```python
from build123d import *

# Parameters (mm, degrees)
EYE_START                  = 22.5
EYE_LUG_SKETCH_R           = 7
EYE_LUG_DEPTH              = 7.5
EYE_START_2                = 2.5
EYE_BOSS_SKETCH_R          = 14
EYE_BOSS_SKETCH_R_2        = 7
EYE_BOSS_28_DEPTH          = 2.5
WEB_RIB_6MM_REACH          = 108.099
WEB_RIB_SKETCH_WALL_W      = 244.198020726
WEB_RIB_SKETCH_WALL_H      = 6
CROSS_BORE_SKETCH_R        = 8
CROSS_BORE_16_DEPTH        = 51.5
TAPPED_HOLE_M12_D          = 10.2
BARREL_SLOT_CUT_DEPTH      = 107.099010428
BARREL_SLOT_CUT_DEPTH_BACK = 107.099010428
BARREL_SLOT_SKETCH_W       = 10
BARREL_SLOT_SKETCH_H       = 8


with BuildPart() as part:
    # Barrel Profile Sketch → Cylinder Barrel (revolve)
    with BuildSketch(Plane.XY, mode=Mode.PRIVATE) as cylinder_barrel_sk:
        Polygon((-39, 11), (-39, 30), (39, 30), (39, 11), (17.5, 11), (17.5, 18), (-17.5, 18), (-17.5, 11), align=None)
    revolve(cylinder_barrel_sk.sketch.rotate(Axis((-46.634042553, 0, 0), (1, 0, 0)), 90), axis=Axis((-46.634042553, 0, 0), (1, 0, 0)))

    # Eye Lug Sketch → Eye Lug (add)
    with BuildSketch(Plane(origin=(0, 0, 0), x_dir=(0, 0, -1), z_dir=(1, 0, 0)).offset(EYE_START)):
        with BuildLine():
            Line((-29.393876913, 6), (-13.71714256, 82.8))
            ThreePointArc((-13.71714256, 82.8), (0, 94), (13.71714256, 82.8))
            Line((13.71714256, 82.8), (29.393876913, 6))
            ThreePointArc((29.393876913, 6), (0, 30), (-29.393876913, 6))
        make_face()
        with Locations((0, 80)):
            Circle(EYE_LUG_SKETCH_R, mode=Mode.SUBTRACT)
    eye_lug = extrude(amount=-EYE_LUG_DEPTH)

    # Eye Boss Sketch → Eye Boss Ø28 (add)
    with BuildSketch(Plane(origin=(22.5, 0, 0), x_dir=(0, 0, -1), z_dir=(1, 0, 0)).offset(EYE_START_2)):
        with Locations(Location((0, 80, 0), (0, 0, 168.463040967))):
            Circle(EYE_BOSS_SKETCH_R)
        with Locations((0, 80)):
            Circle(EYE_BOSS_SKETCH_R_2, mode=Mode.SUBTRACT)
    eye_boss_28 = extrude(amount=-EYE_BOSS_28_DEPTH)

    # Mirrored Eye Lug: Eye Lug, Eye Boss Ø28 across plane
    add(eye_lug.mirror(Plane(origin=(0, 0, 0), x_dir=(0, 0, 1), z_dir=(1, 0, 0))))
    add(eye_boss_28.mirror(Plane(origin=(0, 0, 0), x_dir=(0, 0, 1), z_dir=(1, 0, 0))))

    # Web Rib Sketch wall → Web Rib 6mm (add, up to next)
    with BuildSketch(Plane(origin=(0, 63.7, 0), x_dir=(1, 0, 0), z_dir=(0, 1, 0)), mode=Mode.PRIVATE) as web_rib_6mm_sk1:
        Rectangle(WEB_RIB_SKETCH_WALL_W, WEB_RIB_SKETCH_WALL_H)
    web_rib_6mm_tool1 = extrude(web_rib_6mm_sk1.sketch, amount=-WEB_RIB_6MM_REACH, mode=Mode.PRIVATE) - part.part
    add(web_rib_6mm_tool1.solids().sort_by_distance((0, 63.7, 0))[0])

    # Cross Bore Sketch → Cross Bore Ø16 (cut)
    with BuildSketch(Plane(origin=(0, 0, 0), x_dir=(1, 0, 0), z_dir=(0, 1, 0))):
        with Locations(Location((0, 0, 0), (0, 0, 270))):
            Circle(CROSS_BORE_SKETCH_R)
    extrude(amount=-CROSS_BORE_16_DEPTH, mode=Mode.SUBTRACT)

    # Tapped Hole M12 (through all)
    with Locations(Plane(origin=(0, 46.774811557, 3), x_dir=(1, 0, 0), z_dir=(0, 0, 1))):
        with Locations((0, 0)):
            Hole(TAPPED_HOLE_M12_D / 2)

    # Barrel Slot Sketch → Barrel Slot Cut (cut, two sides: drawn at the far end of the back side and taken through both)
    with BuildSketch(Plane.XY.offset(-BARREL_SLOT_CUT_DEPTH_BACK)):
        with Locations((-34, 26)):
            Rectangle(BARREL_SLOT_SKETCH_W, BARREL_SLOT_SKETCH_H)
        with Locations((34, 26)):
            Rectangle(BARREL_SLOT_SKETCH_W, BARREL_SLOT_SKETCH_H)
    extrude(amount=BARREL_SLOT_CUT_DEPTH + BARREL_SLOT_CUT_DEPTH_BACK, mode=Mode.SUBTRACT)


solid = part.part
```
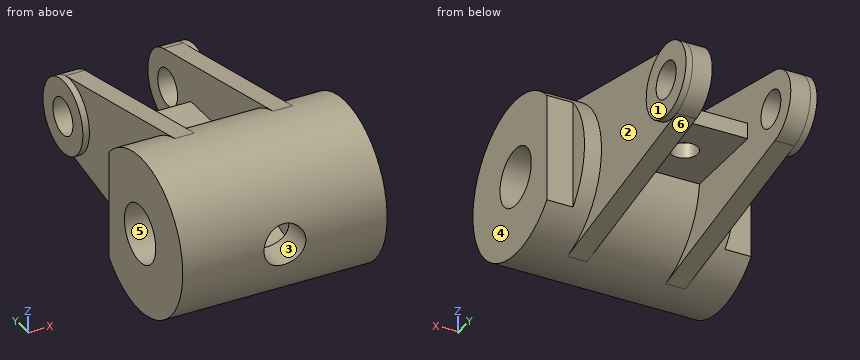
The listing builds one solid part. Answer for the finished solid, in the listing's coordinates (mm). Face numbers are marked on the shaded views. A direction names the side the tool comes from. Coordinates: 2 decimals unless noted, no trailing zeros. Loops run counter-clockwise (first coordinate to the right, second up) from the corner with the lowest first, then second, coordinate; pieces in that order, holes last. Notation, with made-up numbers: (-13.5, -39) -> (23.5, -39) arc R10 ccw to (23.5, -25) -> close; hole circle Ø11 at (26, -17.75). An arc over 180 degrees is marked (long way). Use one line per item in the form item = value. Start each with the question number.
Item 1: A tool of negligible diameter and unlimited length cuts with its end or side. For the marked faces 1, 2 and 3, from which of +Z, -Z, +X, -X, +Y, -Y can it reach the whole face along a straight path? Write none if from no direction.
Item 2: The part is cut by section D-D on x = 11. Determine the outline of the cut face in (y, z), then the cut area to 3 significant figures.
Item 3: The mould has two halves that part along Y. Classify the marked faces 4, 5 and 6: released by +Y, released by -Y, zero draft, split by the parting line, or undercut.
Item 4: Consider L1, parallel to X at y = 76.5, z = -7; L2, parallel to X at y = -22.25, z = 0; L3, parallel to Y at x = 33, z = 0. Determine where each line is inside the solid, lowest interval first. Write a range as [from, to].
Item 5: The part is cut by section B-B on x = 20. Determine the outline of the cut face in (y, z).
Item 6: Flat-ended cylindrical pins translate along their axes: pin 1 Ø1.5 at (x, y) = (12.5, 31) entering from -Z; pin 2 Ø8 at (x, y) = (2.5, -14.5) entering from +Z; pin 3 Ø12 at (y, z) = (36, -18.5) entering from -X; pin 4 Ø8.5 at (y, z) = (80, 0) entering from -X. Find the tip coordinate at first contact, or state that the pin passes through.
Item 7: The part is cut by section A-A on y = 0. Determine the outline of the cut face in (x, z).
Item 8: The part is cut by section C-C on y = 80. Determine the outline of the cut face in (x, z), then the cut area to 3 significant figures.
Answer key:
q1.face_1 = +Z, -Z, +X, +Y
q1.face_2 = +X
q1.face_3 = -Y
q2.outline = (29.85, -3) -> (63.7, -3) -> (63.7, 3) -> (29.85, 3) arc R30 ccw (long way) to start; hole circle Ø36 at (0, 0)
q2.area = 2,010 mm2
q3.face_4 = zero draft
q3.face_5 = undercut
q3.face_6 = released by +Y
q4.L1 = [-25, -15], [15, 25]
q4.L2 = [-39, -8], [8, 39]
q4.L3 = [-30, -11], [11, 22]
q5.outline = (6, -29.39) -> (82.8, -13.72) arc R14 ccw to (82.8, 13.72) -> (6, 29.39) arc R30 ccw (long way) to start; hole circle Ø22 at (0, 0); hole circle Ø14 at (80, 0)
q6.pin_1 = -3
q6.pin_2 = 28.1
q6.pin_3 = -22.5
q6.pin_4 = through
q7.outline = (-39, -30) -> (39, -30) -> (39, -11) -> (17.5, -11) -> (17.5, -18) -> (-17.5, -18) -> (-17.5, -11) -> (-39, -11) -> close; (-39, 11) -> (-17.5, 11) -> (-17.5, 18) -> (17.5, 18) -> (17.5, 11) -> (39, 11) -> (39, 30) -> (-39, 30) -> close
q8.outline = (-25, -14) -> (-22.5, -14) -> (-22.5, -14.29) -> (-15, -14.29) -> (-15, -7) -> (-25, -7) -> close; (-25, 7) -> (-15, 7) -> (-15, 14.29) -> (-22.5, 14.29) -> (-22.5, 14) -> (-25, 14) -> close; (15, -14.29) -> (22.5, -14.29) -> (22.5, -14) -> (25, -14) -> (25, -7) -> (15, -7) -> close; (15, 7) -> (25, 7) -> (25, 14) -> (22.5, 14) -> (22.5, 14.29) -> (15, 14.29) -> close
q8.area = 289 mm2
